Could you check a few things on this model? Use its own coordinates, in mm. Face numbers are marked on the shaded views. A direction names the side the tool comes from. Round coordinates to 2 decimals unless told otherwise and drop trailing zeros. Loops run counter-clockwise (first coordinate to the right, second up) from the corner with the lowest first, then second, coordinate; pieces in that order, holes last. Notation, with made-up numbers: (34.25, -37) -> (87.25, -37) arc R29 cw to (87.25, -12) -> close; hole circle Ø11 at (-9.5, 84). An arc over 180 degrees is marked (long way). One line per item, written item: value.
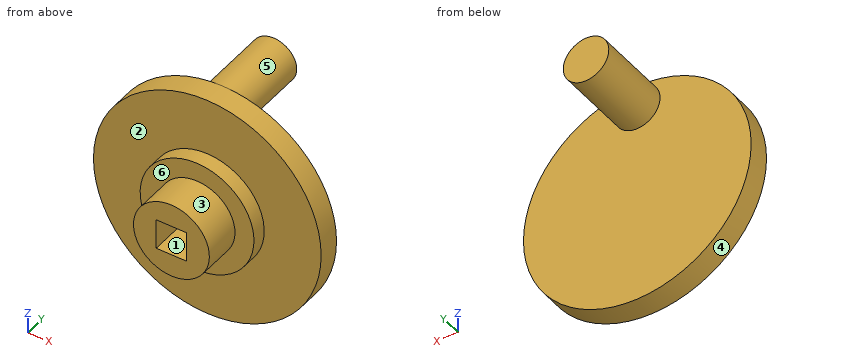
```python
from build123d import *

# Parameters (mm, degrees)
SKETCH1_R           = 15
BOSS_EXTRUDE1_DEPTH = 3
SKETCH2_R           = 3
BOSS_EXTRUDE2_DEPTH = 10
SKETCH3_R           = 5
BOSS_EXTRUDE3_DEPTH = 2
SKETCH4_R           = 5
SKETCH4_W           = 4
SKETCH4_H           = 4
BOSS_EXTRUDE4_DEPTH = 5
SKETCH5_R           = 7.5
BOSS_EXTRUDE5_DEPTH = 2


with BuildPart() as part:
    # Sketch1 → Boss-Extrude1 (new body)
    with BuildSketch(Plane(origin=(0, 0, 0), x_dir=(1, 0, 0), z_dir=(0, 1, 0))):
        with Locations(Location((0, 0, 0), (0, 0, 270))):
            Circle(SKETCH1_R)
    extrude(amount=BOSS_EXTRUDE1_DEPTH)

    # Sketch2 → Boss-Extrude2 (add)
    with BuildSketch(Plane(origin=(0, 3, 0), x_dir=(1, 0, 0), z_dir=(0, 1, 0))):
        with Locations(Location((0, -12, 0), (0, 0, 270))):
            Circle(SKETCH2_R)
    extrude(amount=BOSS_EXTRUDE2_DEPTH)

    # Sketch3 → Boss-Extrude3 (add)
    with BuildSketch(Plane(origin=(0, 0, 0), x_dir=(-1, 0, 0), z_dir=(0, -1, 0))):
        with Locations(Location((0, 0, 0), (0, 0, 90))):
            Circle(SKETCH3_R)
    extrude(amount=BOSS_EXTRUDE3_DEPTH)

    # Sketch4 → Boss-Extrude4 (add)
    with BuildSketch(Plane(origin=(0, -2, 0), x_dir=(-1, 0, 0), z_dir=(0, -1, 0))):
        with Locations(Location((0, 0, 0), (0, 0, 90))):
            Circle(SKETCH4_R)
        Rectangle(SKETCH4_W, SKETCH4_H, mode=Mode.SUBTRACT)
    extrude(amount=BOSS_EXTRUDE4_DEPTH)

    # Sketch5 → Boss-Extrude5 (add)
    with BuildSketch(Plane(origin=(0, 0, 0), x_dir=(-1, 0, 0), z_dir=(0, -1, 0))):
        with Locations(Location((0, 0, 0), (0, 0, 270))):
            Circle(SKETCH5_R)
    extrude(amount=BOSS_EXTRUDE5_DEPTH)


solid = part.part
```
(1) On a 3-axis mill with a long thin cutter (end or side, diameter ignored), from which of +Z, -Z, +X, -X, +Y, -Y can I reach the whole of each face in a straight line? I mean the marked faces 4, 5 and 6. Say none if no direction works.
Results below:
face 4: +Y, -Y
face 5: +Y
face 6: -Y
(2) For pin 1 Ø1.2 at (x, z) = (0.5, 0.5) entering from -Y; pin 2 Ø1.2 at (y, z) = (-5.5, 1) entering from +X; pin 3 Ø15 at (x, z) = (-7.5, -2.5) entering from +Y; pin 4 Ø1.5 at (x, y) = (4.5, 6) entering from +Z, each with a flat end and sliding along its axis, tell me the tip position at first contact or that it passes through.
Results below:
pin 1: stops at y = -2
pin 2: stops at x = 4.98
pin 3: stops at y = 3
pin 4: passes through
(3) Imagine slicing it at C-C on x = 6. Write out the boundary of the cut face in (y, z).
Results below:
outline: (-2, -4.5) -> (0, -4.5) -> (0, -13.75) -> (3, -13.75) -> (3, 13.75) -> (0, 13.75) -> (0, 4.5) -> (-2, 4.5) -> close
(4) Imagine slicing it at D-D on z = 12. Write out the boundary of the cut face in (x, y), then the cut area to 3 significant figures.
Results below:
outline: (-9, 0) -> (9, 0) -> (9, 3) -> (3, 3) -> (3, 13) -> (-3, 13) -> (-3, 3) -> (-9, 3) -> close
area: 114 mm²
(5) We'd pull the mould along Z, two halves only. Please class the marked faces 1, 2 and 3: +Z half, -Z half, draft (parallel to the pull), parting line (faces both ways), or undercut.
Results below:
face 1: undercut
face 2: draft
face 3: parting line
(6) Please list where these lines run through material, in increasing order: L1, parallel to X at y = -5.75, z = 0; L2, parallel to Y at x = -3.75, z = -5.5; L3, parallel to Y at x = -4, z = 2.25.
Results below:
L1: x = -5 to -2, 2 to 5
L2: y = -2 to 3
L3: y = -7 to 3
(7) Imagine slicing it at A-A on z = 0. Write out the boundary of the cut face in (x, y), then the cut area to 3 significant figures.
Results below:
outline: (-15, 0) -> (-7.5, 0) -> (-7.5, -2) -> (-5, -2) -> (-5, -7) -> (-2, -7) -> (-2, -2) -> (2, -2) -> (2, -7) -> (5, -7) -> (5, -2) -> (7.5, -2) -> (7.5, 0) -> (15, 0) -> (15, 3) -> (-15, 3) -> close
area: 150 mm²
(8) Imagine slicing it at B-B on y = -2.75. Write out the boundary of the cut face in (x, z), then the cut area to 3 significant figures.
Results below:
outline: circle Ø10 at (0, 0); hole (-2, -2) -> (2, -2) -> (2, 2) -> (-2, 2) -> close
area: 62.5 mm²
